For this review, take the finished solid that the model builds, in its own axes (mm). Face numbers are marked on the shaded views. A direction names the side the tool comes from. Coordinates: 2 decimals unless noted, no trailing zeros. Order: outer loops, then holes, each group sorted by start corner. A loop starts at its lowest first (then second) coordinate and runs counter-clockwise, first axis right, second up. Notation, with made-up numbers: M 58,6.25 L 98,6.25 A13 ccw 98,18.25 Z; hole C 37,-24.75 d2. An arc over 180 degrees is marked long. Use CSV: the item, a comma, the result in double quotes.
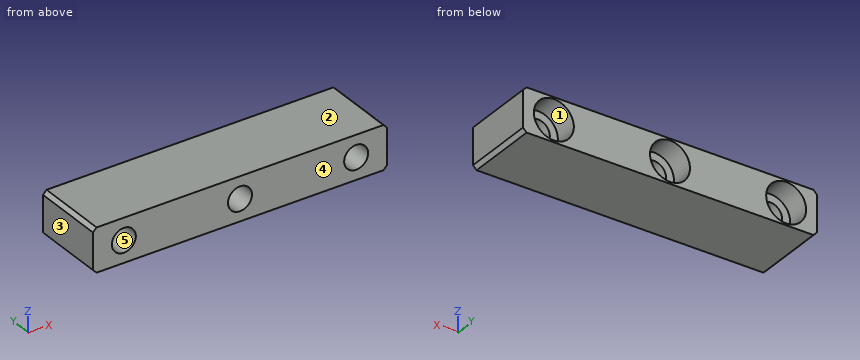
```python
from build123d import *

# Parameters (mm, degrees)
SKETCH_1_W                   = 81
SKETCH_1_H                   = 20
EXTRUDE_1_DEPTH              = 12
HOLE_WIZARD_M6_1_D           = 6.6
HOLE_WIZARD_M6_1_CBORE_D     = 11
HOLE_WIZARD_M6_1_CBORE_DEPTH = 6.4
CHAMFER_1_SIZE               = 1


with BuildPart() as part:
    # 草图1 → 凸台-拉伸1 (new body)
    with BuildSketch(Plane.XY):
        Rectangle(SKETCH_1_W, SKETCH_1_H)
    extrude(amount=EXTRUDE_1_DEPTH)

    # M6 六角凹头螺钉的柱形沉头孔1 (through all)
    with Locations(Plane(origin=(0, 10, 0), x_dir=(1, 0, 0), z_dir=(0, 1, 0))):
        with Locations((-32, -6), (0, -6), (32, -6)):
            CounterBoreHole(HOLE_WIZARD_M6_1_D / 2, HOLE_WIZARD_M6_1_CBORE_D / 2, HOLE_WIZARD_M6_1_CBORE_DEPTH)

    # 倒角1
    chamfer_1_edges = [part.edges().sort_by_distance(p)[0] for p in [
        (-40.5, 0, 12),
        (40.5, 0, 12),
        (-40.5, 0, 0),
        (40.5, 0, 0),
    ]]
    chamfer(chamfer_1_edges, length=CHAMFER_1_SIZE)


solid = part.part
```
Item 1: Add section A-A on z = 6. State the section outline as (x, y) points, and give its area (3 significant figures).
Solutions:
outline,"M -40.5,-10 L -35.3,-10 L -35.3,3.6 L -37.5,3.6 L -37.5,10 L -40.5,10 Z; M -28.7,-10 L -3.3,-10 L -3.3,3.6 L -5.5,3.6 L -5.5,10 L -26.5,10 L -26.5,3.6 L -28.7,3.6 Z; M 3.3,-10 L 28.7,-10 L 28.7,3.6 L 26.5,3.6 L 26.5,10 L 5.5,10 L 5.5,3.6 L 3.3,3.6 Z; M 35.3,-10 L 40.5,-10 L 40.5,10 L 37.5,10 L 37.5,3.6 L 35.3,3.6 Z"
area,"1,140 mm^2"
Item 2: Add section C-C on x = 0. State the section outline as (y, z) points, and give its area (3 significant figures).
Solutions:
outline,"M -10,0 L 10,0 L 10,0.5 L 3.6,0.5 L 3.6,2.7 L -10,2.7 Z; M -10,9.3 L 3.6,9.3 L 3.6,11.5 L 10,11.5 L 10,12 L -10,12 Z"
area,"79.8 mm^2"
Item 3: Clearance check with flat-ended pins moving along their axes: pin 1 Ø4 at (x, z) = (-32, 6) entering from +Y; pin 2 Ø3.5 at (x, z) = (-32.5, 4.5) entering from +Y. State where each tip first meets the part, or that it passes through.
Solutions:
pin 1,"through"
pin 2,"y = 3.6"
Item 4: Add section B-B on y = -4.75. State the section outline as (x, z) points, and give its area (3 significant figures).
Solutions:
outline,"M -40.5,1 L -39.5,0 L 39.5,0 L 40.5,1 L 40.5,11 L 39.5,12 L -39.5,12 L -40.5,11 Z; hole C -32,6 d6.6; hole C 0,6 d6.6; hole C 32,6 d6.6"
area,"867 mm^2"
Item 5: For the marked faces 1 and 2, list the 3-axis set-ups (+Z, -Z, +X, -X, +Y, -Y) from which the entire face can be reached by the end or side of a thin tool; tool diameter is ignored.
Solutions:
face 1,"+Y"
face 2,"+Z, +X, -X, +Y, -Y"
Item 6: Draft analysis for pull direction X (two halves, no side actions). For the marked faces 3, 4 and 5, state which applies: released by +X, released by -X, zero draft, split by the parting line, or undercut.
Solutions:
face 3,"released by -X"
face 4,"zero draft"
face 5,"undercut"
Item 7: To check wall thickness, follow line 1 along Z through (x, y) = (0, 7); line 2 along X through (y, z) = (8, 2.25); line 3 along Z through (x, y) = (32, -6.5). State the ranges of each line that lie inside material, in increasing order. Write a range as [from, to].
Solutions:
line 1,"[0, 0.5], [11.5, 12]"
line 2,"[-40.5, -36.02], [-27.98, -4.02], [4.02, 27.98], [36.02, 40.5]"
line 3,"[0, 2.7], [9.3, 12]"
